Build history of the part. All positions in model axes, mm. Face numbers are marked on the shaded views. A direction names the side the tool comes from. Round coordinates to 2 decimals unless told otherwise and drop trailing zeros. Order: outer loops, then holes, each group sorted by start corner. A loop starts at its lowest first (then second) coordinate and runs counter-clockwise, first axis right, second up. Notation, with made-up numbers: (30.5, 45) -> (57.5, 45) arc R25 ccw to (57.5, 83) -> close; hole circle Ø10 at (-20.5, 50). An arc over 180 degrees is marked (long way). Use a Markdown table: item, result. Add a question column.
Item 1: Slice it at A-A, the plane z = 28.5. Give the cut face in (x, y).
Item 2: Probe L1, parallel to Y at x = 140, z = -1.5; L2, parallel to Y at x = 38, z = -36; L3, parallel to Y at x = 25.5, z = 6. List the from-to ranges inside material, lowest first.
Item 3: 3-axis set-ups, long thin cutter, end or side, ignore diameter. For the marked faces 1, 2 and 3: which of +Z, -Z, +X, -X, +Y, -Y reach the whole face in a straight line?
Item 4: Slice it at B-B, the plane x = 35. Give the cut face in (y, z), plus the area to 3 significant figures.
Item 5: Pin check, flat tips, straight feed: pin 1 (1.5 mm diameter, centred on y = 16.5, z = 17.5, fed in from +X); pin 2 (10 mm diameter, centred on x = 14.5, y = 11, fed in from -Z); pin 3 (1.5 mm diameter, centred on x = 104.5, z = -3, fed in from +Y). Stop position of each tip, or through.
Item 6: Two-plate mould, pull along Y, no slides. Class the marked faces 4, 5 and 6: released by +Y, released by -Y, zero draft, split by the parting line, or undercut.
Item 7: Slice it at D-D, the plane y = 32. Give the cut face in (x, z), plus the area to 3 significant figures.
Item 8: Slice it at C-C, the plane z = 1. Give the cut face in (x, y).
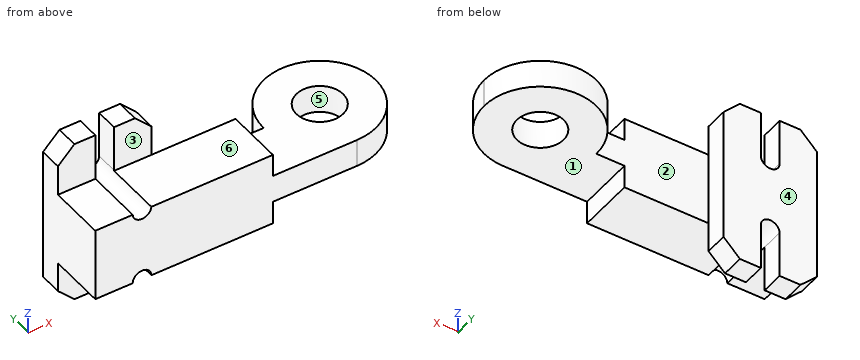
from build123d import *

# Parameters (mm, degrees)
BASE_BODY_42MM_DEPTH = 42
SKETCH1_5_W          = 15
SKETCH1_5_H          = 15
SIDE_BOSS_30MM_DEPTH = 30
SLOTS_SKETCH_W       = 16.483923251
SLOTS_SKETCH_H       = 30
SLOTS_SKETCH_W_2     = 8.802682669
SLOTS_SKETCH_W_3     = 16.197317331
SLOTS_CUT_DEPTH      = 123
SKETCH1_6_W          = 30
SKETCH1_6_H          = 15
EYE_BOSS_70MM_DEPTH  = 70
WEB_SKETCH_W         = 30
WEB_SKETCH_H         = 15
WEB_BOSS_70MM_DEPTH  = 70
PIN_BORE_SKETCH_R    = 12.5
PIN_BORE_CUT_DEPTH   = 15


with BuildPart() as part:
    # Link Profile Sketch → Base Body 42mm (new body)
    with BuildSketch(Plane(origin=(0, 0, 0), x_dir=(1, 0, 0), z_dir=(0, 1, 0))):
        with BuildLine():
            Line((20, -20), (20, -45))
            Line((20, -45), (8.802682669, -45))
            Line((8.802682669, -45), (0, -36.197317331))
            Line((0, -36.197317331), (0, 0))
            Line((0, 0), (0, 36.197317331))
            Line((0, 36.197317331), (8.802682669, 45))
            Line((8.802682669, 45), (20, 45))
            Line((20, 45), (20, 20))
            ThreePointArc((20, 20), (25, 15), (30, 20))
            Line((30, 20), (30, 45))
            Line((30, 45), (41.197317331, 45))
            Line((41.197317331, 45), (50, 36.197317331))
            Line((50, 36.197317331), (50, -36.197317331))
            Line((50, -36.197317331), (41.197317331, -45))
            Line((41.197317331, -45), (30, -45))
            Line((30, -45), (30, -20))
            ThreePointArc((30, -20), (25, -15), (20, -20))
        make_face()
    extrude(amount=BASE_BODY_42MM_DEPTH)

    # Sketch1_5 → Side Boss 30mm (add)
    with BuildSketch(Plane(origin=(0, 0, 0), x_dir=(1, 0, 0), z_dir=(0, 1, 0))):
        Polygon((95, 20), (50, 20), (50, -20), (95, -20), (95, -7.5), (95, 7.5), align=None)
        with Locations((102.5, 0)):
            Rectangle(SKETCH1_5_W, SKETCH1_5_H)
    extrude(amount=SIDE_BOSS_30MM_DEPTH)

    # Slots Sketch → Slots Cut (cut)
    with BuildSketch(Plane.ZY):
        with Locations((27.955355706, 15)):
            Rectangle(SLOTS_SKETCH_W, SLOTS_SKETCH_H)
        with Locations((40.598658665, 15)):
            Rectangle(SLOTS_SKETCH_W_2, SLOTS_SKETCH_H)
        with Locations((-28.098658666, 15)):
            Rectangle(SLOTS_SKETCH_W_3, SLOTS_SKETCH_H)
        with Locations((-40.598658665, 15)):
            Rectangle(SLOTS_SKETCH_W_2, SLOTS_SKETCH_H)
    extrude(amount=-SLOTS_CUT_DEPTH, mode=Mode.SUBTRACT)

    # Sketch1_6 → Eye Boss 70mm (add)
    with BuildSketch(Plane(origin=(0, 0, 0), x_dir=(1, 0, 0), z_dir=(0, 1, 0))):
        with Locations((125, 0)):
            Rectangle(SKETCH1_6_W, SKETCH1_6_H)
    extrude(amount=EYE_BOSS_70MM_DEPTH)

    # Web Sketch → Web Boss 70mm (add)
    with BuildSketch(Plane(origin=(0, 70, 0), x_dir=(1, 0, 0), z_dir=(0, 1, 0))):
        with Locations((155, 0)):
            Rectangle(WEB_SKETCH_W, WEB_SKETCH_H)
    extrude(amount=-WEB_BOSS_70MM_DEPTH)

    # Pin Bore Sketch → Pin Bore Cut (cut)
    with BuildSketch(Plane.XY.offset(7.5)):
        with Locations((140, 30)):
            Circle(PIN_BORE_SKETCH_R)
        with BuildLine():
            Line((110, 70), (110, 30))
            ThreePointArc((110, 30), (140, 60), (170, 30))
            Line((170, 30), (170, 70))
            Line((170, 70), (110, 70))
        make_face()
        with BuildLine():
            Line((170, 0), (170, 30))
            ThreePointArc((170, 30), (161.213203436, 8.786796564), (140, 0))
            Line((140, 0), (170, 0))
        make_face()
    extrude(amount=-PIN_BORE_CUT_DEPTH, mode=Mode.SUBTRACT)


solid = part.part
Check sheet entries:
| question | item | result |
|---|---|---|
| 1 | outline | (0, 30) -> (20, 30) -> (20, 42) -> (0, 42) -> close; (30, 30) -> (50, 30) -> (50, 42) -> (30, 42) -> close |
| 2 | L1 | 0 to 17.5, 42.5 to 60 |
| 2 | L2 | 30 to 42 |
| 2 | L3 | 0 to 42 |
| 3 | face 1 | -Z, +X, +Y, -Y |
| 3 | face 2 | +Z, -Z, +Y |
| 3 | face 3 | +Z, +X, -X, -Y |
| 4 | outline | (0, -20) -> (30, -20) -> (30, -45) -> (42, -45) -> (42, 45) -> (30, 45) -> (30, 19.71) -> (0, 19.71) -> close |
| 4 | area | 2,270 mm2 |
| 5 | pin 1 | x = 95 |
| 5 | pin 2 | z = -20 |
| 5 | pin 3 | y = 30 |
| 6 | face 4 | released by +Y |
| 6 | face 5 | undercut |
| 6 | face 6 | zero draft |
| 7 | outline | (0, -36.2) -> (8.8, -45) -> (20, -45) -> (20, -20) arc R5 cw to (30, -20) -> (30, -45) -> (41.2, -45) -> (50, -36.2) -> (50, 36.2) -> (41.2, 45) -> (30, 45) -> (30, 20) arc R5 cw to (20, 20) -> (20, 45) -> (8.8, 45) -> (0, 36.2) -> close; (110.07, -7.5) -> (127.66, -7.5) -> (127.66, 7.5) -> (110.07, 7.5) -> close; (152.34, -7.5) -> (169.93, -7.5) -> (169.93, 7.5) -> (152.34, 7.5) -> close |
| 7 | area | 4,290 mm2 |
| 8 | outline | (0, 0) -> (140, 0) arc R30 ccw (long way) to (110, 30) -> (50, 30) -> (50, 42) -> (0, 42) -> close; hole circle Ø25 at (140, 30) |
